Geometry check sheet. Reference: the model listing, model coordinates, mm. Face numbers are marked on the shaded views. A direction names the side the tool comes from. Coordinates: 2 decimals unless noted, no trailing zeros. Write each loop counter-clockwise with the first axis right and the second up, starting at its lowest first coordinate (ties: lowest second). Pieces come first, ordered by that corner, then holes.
from build123d import *

# Parameters (mm, degrees)
BOSS_EXTRUDE1_DEPTH = 22.5
SKETCH3_R           = 18
BOSS_EXTRUDE2_DEPTH = 260
CHAMFER1_SIZE       = 3.6


with BuildPart() as part:
    # Sketch1 → Boss-Extrude1 (new body)
    with BuildSketch(Plane.XY):
        Polygon((27.5, 15.877132403), (0, 31.754264805), (-27.5, 15.877132403), (-27.5, -15.877132403), (0, -31.754264805), (27.5, -15.877132403), align=None)
    extrude(amount=BOSS_EXTRUDE1_DEPTH)

    # Sketch3 → Boss-Extrude2 (add)
    with BuildSketch(Plane.XY.offset(22.5)):
        Circle(SKETCH3_R)
    extrude(amount=BOSS_EXTRUDE2_DEPTH)

    # Chamfer1
    chamfer1_edges = [part.edges().sort_by_distance(p)[0] for p in [
        (-18, 0, 282.5),
    ]]
    chamfer(chamfer1_edges, length=CHAMFER1_SIZE)


solid = part.part
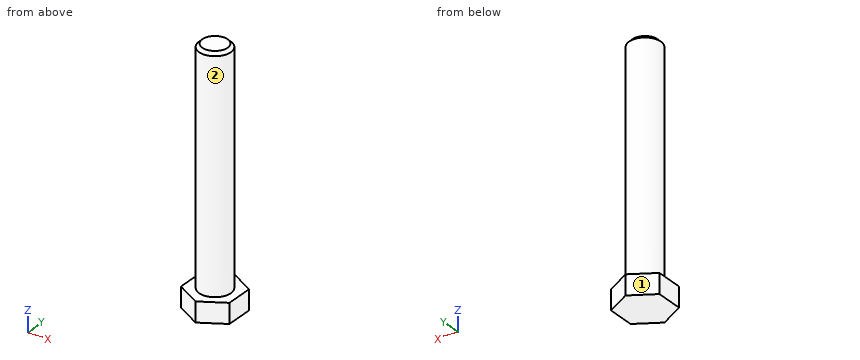
1. Sectioned sample at C-C, the plane y = -25. Record the boundary of the cut face in (x, z), and give its area (3 significant figures).
Computed values:
outline: (-11.7, 0) - (11.7, 0) - (11.7, 22.5) - (-11.7, 22.5) - close
area: 526 mm2
2. Gauge pin test, flat ends, axial feed: pin 1 Ø10 at (y, z) = (-7, 77.5) entering from -X; pin 2 Ø2 at (x, z) = (-20, 46) entering from +Y; pin 3 Ø1.5 at (x, z) = (-16, 196) entering from +Y; pin 4 Ø10 at (y, z) = (12, 227.5) entering from -X. Record the tip position at first contact, or that the pin passes through.
Computed values:
pin 1: stops at x = -17.89
pin 2: passes through
pin 3: stops at y = 9.56
pin 4: stops at x = -16.58
3. Sectioned sample at B-B, the plane z = 139. Record the boundary of the cut face in (x, y).
Computed values:
outline: circle Ø36 at (0, 0)
4. Sectioned sample at A-A, the plane y = 0. Record the boundary of the cut face in (x, z), and give its area (3 significant figures).
Computed values:
outline: (-27.5, 0) - (27.5, 0) - (27.5, 22.5) - (18, 22.5) - (18, 278.9) - (14.4, 282.5) - (-14.4, 282.5) - (-18, 278.9) - (-18, 22.5) - (-27.5, 22.5) - close
area: 10,600 mm2
5. Access from +Z, -Z, +X, -X, +Y, -Y to the whole of each face (thin tool, end or side, straight path). Record for the marked faces 1 and 2.
Computed values:
face 1: +Z, -Z, -X, +Y
face 2: +Z
6. Thickness scan on line 1 along Z through (x, y) = (-14, -16.5); line 2 along Y through (x, z) = (0.5, 204); line 3 along X through (y, z) = (8.5, 115). Record the ranges inside material, lowest first.
Computed values:
line 1: z = 0 to 22.5
line 2: y = -17.99 to 17.99
line 3: x = -15.87 to 15.87
